Can you work these out from the drawing? Everything is in mm from the part's minimum corner. A direction names the side the tool comes from. Coordinates: 2 decimals unless noted, no trailing zeros. Write each loop counter-clockwise with the first axis right and the second up, starting at its lowest first coordinate (ties: lowest second). Pieces come first, ordered by that corner, then holes. Notation, with made-up numbers: (-16.5, 4) -> (26.5, 4) arc R23 ccw to (26.5, 39) -> close; hole circle Ø5 at (8.25, 65.25). An arc over 180 degrees is marked (long way). Use CSV: the item, a comma, the result in double quotes. Start each with the question number.
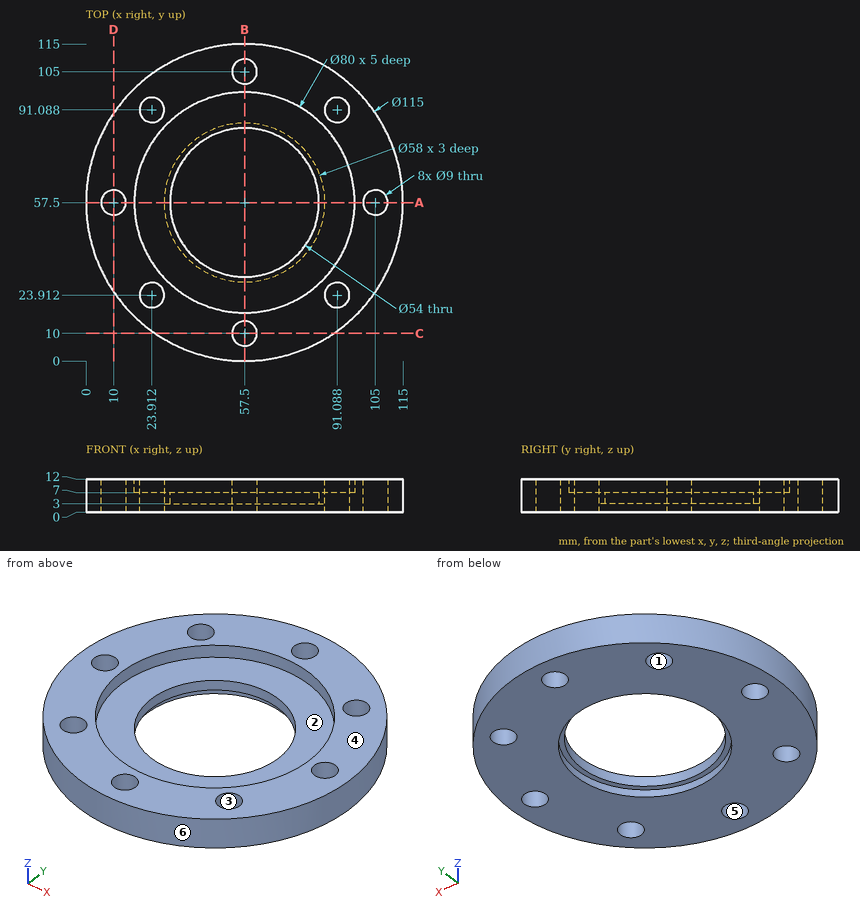
Item 1: Which directions (+Z, -Z, +X, -X, +Y, -Y) give clear straight access to the entire face, cutting with the end or side of a thin tool? Please do the marked faces 1 and 2.
Item 2: I want a section at C-C on y = 10. Please give me the cut outline in (x, z), then the cut area to 3 significant figures.
Item 3: Thinking about a two-plate mould opening in X: for the marked faces 3, 4, 5 and 6, which applies, +X half, -X half, draft (parallel to the pull), parting line (faces both ways), or undercut?
Item 4: If I drill on line 1 along Y through (x, z) = (57.5, 2.45); line 2 along Y through (x, z) = (57.5, 5.25); line 3 along X through (y, z) = (57, 11.25), over which ranges is the centre line in solid material (lowest first)?
Item 5: I want a section at A-A on y = 57.5. Please give me the cut outline in (x, z).
Item 6: I'm going to push flat-ended pins straight in: pin 1 (10.5 mm diameter, centred on x = 23.91, y = 23.91, fed in from -Z); pin 2 (6 mm diameter, centred on x = 52, z = 10, fed in from -Y); pin 3 (3 mm diameter, centred on y = 70, z = 3, fed in from -X); pin 4 (6 mm diameter, centred on y = 49, z = 6, fed in from +X). Where does each tip first touch, or does it pass through?
Geometry says:
1,face 1,"+Z, -Z"
1,face 2,"+Z"
2,outline,"(25.1, 0) -> (53, 0) -> (53, 12) -> (25.1, 12) -> close; (62, 0) -> (89.9, 0) -> (89.9, 12) -> (62, 12) -> close"
2,area,"670 mm2"
3,face 3,"undercut"
3,face 4,"draft"
3,face 5,"undercut"
3,face 6,"parting line"
4,line 1,"0 to 5.5, 14.5 to 28.5, 86.5 to 100.5, 109.5 to 115"
4,line 2,"0 to 5.5, 14.5 to 30.5, 84.5 to 100.5, 109.5 to 115"
4,line 3,"0 to 5.53, 14.47 to 17.5, 97.5 to 100.53, 109.47 to 115"
5,outline,"(0, 0) -> (5.5, 0) -> (5.5, 12) -> (0, 12) -> close; (14.5, 0) -> (28.5, 0) -> (28.5, 3) -> (30.5, 3) -> (30.5, 7) -> (17.5, 7) -> (17.5, 12) -> (14.5, 12) -> close; (84.5, 3) -> (86.5, 3) -> (86.5, 0) -> (100.5, 0) -> (100.5, 12) -> (97.5, 12) -> (97.5, 7) -> (84.5, 7) -> close; (109.5, 0) -> (115, 0) -> (115, 12) -> (109.5, 12) -> close"
6,pin 1,"z = 0"
6,pin 2,"y = 0.05"
6,pin 3,"x = 1.06"
6,pin 4,"x = 114.74"
